```python
from build123d import *

# Parameters (mm, degrees)
SKETCH_1_W      = 745
SKETCH_1_H      = 1196
EXTRUDE_1_DEPTH = 22
SHELL_1_T       = -2
SKETCH_2_W      = 745
SKETCH_2_H      = 1196
SKETCH_2_W_2    = 705
SKETCH_2_H_2    = 1156
EXTRUDE_2_DEPTH = 2


with BuildPart() as part:
    # 草图1 → 凸台-拉伸1 (new body)
    with BuildSketch(Plane.XY):
        with Locations((372.5, 598)):
            Rectangle(SKETCH_1_W, SKETCH_1_H)
    extrude(amount=EXTRUDE_1_DEPTH)

    # 抽壳1
    shell_1_openings = [part.faces().sort_by_distance(p)[0] for p in [
        (372.5, 598, 22),
    ]]
    offset(amount=SHELL_1_T, openings=shell_1_openings, kind=Kind.INTERSECTION)

    # 草图2 → 凸台-拉伸2 (add)
    with BuildSketch(Plane.XY.offset(22)):
        with Locations((372.5, 598)):
            Rectangle(SKETCH_2_W, SKETCH_2_H)
        with Locations((372.5, 598)):
            Rectangle(SKETCH_2_W_2, SKETCH_2_H_2, mode=Mode.SUBTRACT)
    extrude(amount=-EXTRUDE_2_DEPTH)


solid = part.part
```
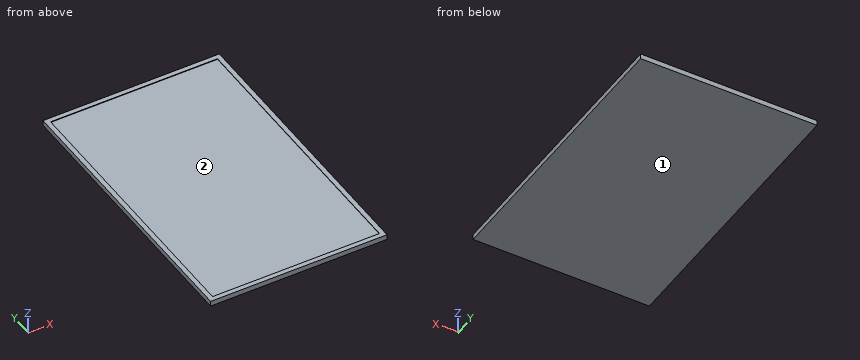
Build history of the part. All positions in model axes, mm. Face numbers are marked on the shaded views. Give positions to 0.01 mm unless a question says otherwise; leave off trailing zeros. Loops run counter-clockwise (first coordinate to the right, second up) from the corner with the lowest first, then second, coordinate; pieces in that order, holes last. Notation, with made-up numbers: (-24, 2.25) -> (-20, 2.25) arc R23 cw to (-20, 14.25) -> close; hole circle Ø7 at (-40, -36). An arc over 180 degrees is marked (long way). One line per question, with ' | ' between items. Start each with the question number.
1) Probe L1, parallel to Y at x = 464.5, z = 3.25; L2, parallel to X at y = 886.5, z = 12.5; L3, parallel to X at y = 1087.5, z = 21. List the from-to ranges inside material, lowest first.
2) Cut at A-A (z = 15.5). Give the cut face in (x, y), plus the area to 3 significant figures.
3) Cut at C-C (y = 771). Give the cut face in (x, z), plus the area to 3 significant figures.
4) Cut at B-B (x = 515). Give the cut face in (y, z), plus the area to 3 significant figures.
5) Pin check, flat tip, straight feed: pin 1 (12 mm diameter, centred on x = 570, y = 504.5, fed in from +Z). Stop position of the tip, or through.
6) Two-plate mould, pull along Y, no slides. Class the marked faces 1 and 2: released by +Y, released by -Y, zero draft, split by the parting line, or undercut.
Return value:
1) L1: 0 to 2, 1194 to 1196 | L2: 0 to 2, 743 to 745 | L3: 0 to 20, 725 to 745
2) outline: (0, 0) -> (745, 0) -> (745, 1196) -> (0, 1196) -> close; hole (2, 2) -> (743, 2) -> (743, 1194) -> (2, 1194) -> close | area: 7,750 mm^2
3) outline: (0, 0) -> (745, 0) -> (745, 22) -> (725, 22) -> (725, 20) -> (743, 20) -> (743, 2) -> (2, 2) -> (2, 20) -> (20, 20) -> (20, 22) -> (0, 22) -> close | area: 1,640 mm^2
4) outline: (0, 0) -> (1196, 0) -> (1196, 22) -> (1176, 22) -> (1176, 20) -> (1194, 20) -> (1194, 2) -> (2, 2) -> (2, 20) -> (20, 20) -> (20, 22) -> (0, 22) -> close | area: 2,540 mm^2
5) pin 1: z = 2
6) face 1: zero draft | face 2: undercut
